The model under review builds one solid part; all positions refer to its coordinate system, in mm. A direction names the side the tool comes from. Round coordinates to 2 decimals unless told otherwise and drop trailing zeros. Order: outer loops, then holes, each group sorted by start corner. A loop starts at its lowest first (then second) coordinate and runs counter-clockwise, first axis right, second up.
1) Clearance check with flat-ended pins moving along their axes: P1, Ø4, axis at x = -2.5, y = -13, coming from the +Z side; P2, Ø5, axis at x = 3, y = -13, coming from the +Z side; P3, Ø3, axis at x = 6, z = 5.2, coming from the -Y side. State where each tip first meets the part, or that it passes through.
2) Consider section B-B (z = 5.2). Give the boundary of the cut face in (x, y), then the cut area to 3 significant figures.
3) Consider section C-C (y = 17.5). Give the boundary of the cut face in (x, z), then the cut area to 3 significant figures.
4) Consider section D-D (x = -14.5). Give the boundary of the cut face in (y, z), then the cut area to 3 significant figures.
5) Machinability: for faces 1 (the face through (5, -9, 0)), 2 (the face through (0, -15.2, 6)), 3 (the face through (4.78, 18.3, 5.47)), 4 (the face through (-0.2, 15.5, 7.7)), which of the approach directions +Z, -Z, +X, -X, +Y, -Y give a long, thin tool a straight path to every point of the face, cutting with its end or side? Answer none if there is none.
6) Mouldability with a two-part tool opening along X and no side actions: class faces 5 (the face through (0.2, -15.4, 7.7)), 6 (the face through (20.32, -8.43, 1.76)), 7 (the face through (0, 15.2, 6)) as pulls with the +X half, pulls with the -X half, needs draft (parallel to the pull), parting line crosses it, or undercut.
7) Consider section A-A (z = 9.25). Give the boundary of the cut face in (x, y).
8) To check wall thickness, follow L1, parallel to Y at x = 0, z = 3; L2, parallel to Y at x = 0, z = 2; L3, parallel to Z at x = 6, y = 19. State the ranges of each line that lie inside material, in increasing order.
from build123d import *

# Parameters (mm, degrees)
SKETCH1_R           = 22
BOSS_EXTRUDE1_DEPTH = 11
SKETCH2_R           = 20.05
CUT_EXTRUDE1_DEPTH  = 8.3
SKETCH3_W           = 67.682797152
SKETCH3_H           = 30.4
CUT_EXTRUDE2_DEPTH  = 8.3
SKETCH4_R           = 1.75
CUT_EXTRUDE3_DEPTH  = 5
CIRPATTERN1_COUNT   = 2
CUT_EXTRUDE4_REACH  = 35
SKETCH5_R           = 9
CHAMFER1_SIZE       = 1.5
CHAMFER2_SIZE       = 0.5
SKETCH6_OUTSIDE_W   = 58.638
SKETCH6_OUTSIDE_H   = 58.638
SKETCH6_OUTSIDE_W_2 = 90.952157774
SKETCH6_OUTSIDE_H_2 = 47
CUT_EXTRUDE5_DEPTH  = 8.3
BOSS_EXTRUDE2_START = 5
SKETCH7_R           = 1.75
BOSS_EXTRUDE2_DEPTH = 5
SKETCH8_R           = 1.25
CUT_EXTRUDE6_DEPTH  = 11


with BuildPart() as part:
    # Sketch1 → Boss-Extrude1 (new body)
    with BuildSketch(Plane.XY):
        Circle(SKETCH1_R)
    extrude(amount=BOSS_EXTRUDE1_DEPTH)

    # Sketch2 → Cut-Extrude1 (cut)
    with BuildSketch(Plane.XY.offset(11)):
        Circle(SKETCH2_R)
    extrude(amount=-CUT_EXTRUDE1_DEPTH, mode=Mode.SUBTRACT)

    # Sketch3 → Cut-Extrude2 (cut)
    with BuildSketch(Plane.XY.offset(2.7)):
        Rectangle(SKETCH3_W, SKETCH3_H)
    extrude(amount=CUT_EXTRUDE2_DEPTH, mode=Mode.SUBTRACT)

    # Sketch4 → Cut-Extrude3 (cut)
    with BuildSketch(Plane(origin=(0, 0, 0), x_dir=(-1, 0, 0), z_dir=(0, 0, -1))):
        with Locations((0, 17.5)):
            Circle(SKETCH4_R)
    cut_extrude3 = extrude(amount=-CUT_EXTRUDE3_DEPTH, mode=Mode.SUBTRACT)

    # CirPattern1: Cut-Extrude3 ×2 about axis
    cirpattern1_axis = Axis((0, 0, 0), (0, 0, 1))
    for i in range(1, CIRPATTERN1_COUNT):
        add(cut_extrude3.rotate(cirpattern1_axis, i * 360 / CIRPATTERN1_COUNT), mode=Mode.SUBTRACT)

    # Sketch5 → Cut-Extrude4 (cut, up to next)
    with BuildSketch(Plane(origin=(0, 0, 0), x_dir=(-1, 0, 0), z_dir=(0, 0, -1)), mode=Mode.PRIVATE) as cut_extrude4_sk1:
        Circle(SKETCH5_R)
    cut_extrude4_tool1 = extrude(cut_extrude4_sk1.sketch, amount=-CUT_EXTRUDE4_REACH, mode=Mode.PRIVATE) & part.part
    add(cut_extrude4_tool1.solids().sort_by_distance((0, 0, 0))[0], mode=Mode.SUBTRACT)

    # Chamfer1
    chamfer1_edges = [part.edges().sort_by_distance(p)[0] for p in [
        (1.75, 17.5, 0),
        (-1.75, -17.5, 0),
    ]]
    chamfer(chamfer1_edges, length=CHAMFER1_SIZE)

    # Chamfer2
    chamfer2_edges = [part.edges().sort_by_distance(p)[0] for p in [
        (9, 0, 0),
    ]]
    chamfer(chamfer2_edges, length=CHAMFER2_SIZE)

    # Sketch6 outside → Cut-Extrude5 (cut)
    with BuildSketch(Plane.XY.offset(11)):
        Rectangle(SKETCH6_OUTSIDE_W, SKETCH6_OUTSIDE_H)
        Rectangle(SKETCH6_OUTSIDE_W_2, SKETCH6_OUTSIDE_H_2, mode=Mode.SUBTRACT)
    extrude(amount=-CUT_EXTRUDE5_DEPTH, mode=Mode.SUBTRACT)

    # Sketch7 → Boss-Extrude2 (add)
    # profile 1 of 2: a face of its own
    with BuildSketch(Plane.XY.offset(2.7).offset(BOSS_EXTRUDE2_START)):
        with BuildLine():
            Line((-13.075262904, 15.2), (13.075262904, 15.2))
            ThreePointArc((13.075262904, 15.2), (0, 20.05), (-13.075262904, 15.2))
        make_face()
        with Locations((0, 17.5)):
            Circle(SKETCH7_R, mode=Mode.SUBTRACT)
    # profile 2 of 2: a face of its own
    with BuildSketch(Plane.XY.offset(2.7).offset(BOSS_EXTRUDE2_START)):
        with BuildLine():
            Line((-13.075262904, -15.2), (13.075262904, -15.2))
            ThreePointArc((13.075262904, -15.2), (0, -20.05), (-13.075262904, -15.2))
        make_face()
        with Locations((0, -17.5)):
            Circle(SKETCH7_R, mode=Mode.SUBTRACT)
    extrude(amount=-BOSS_EXTRUDE2_DEPTH)

    # Sketch8 → Cut-Extrude6 (cut)
    with BuildSketch(Plane.XZ.offset(-15.2)):
        with Locations(Location((6, 5.2, 0), (0, 0, 270))):
            Circle(SKETCH8_R)
    extrude(amount=-CUT_EXTRUDE6_DEPTH, mode=Mode.SUBTRACT)


solid = part.part
Answer below:
1. P1: stops at z = 2.7
1. P2: stops at z = 7.7
1. P3: stops at y = -21.53
2. outline: (-15.9, -15.2) arc R22 ccw to (15.9, -15.2) - close; (-15.9, 15.2) - (4.75, 15.2) - (4.75, 21.48) arc R22 ccw to start; (7.25, 15.2) - (15.9, 15.2) arc R22 ccw to (7.25, 20.77) - close; hole circle Ø3.5 at (0, -17.5); hole circle Ø3.5 at (0, 17.5)
2. area: 265 mm2
3. outline: (-13.33, 0) - (-3.25, 0) - (-1.75, 1.5) - (-1.75, 7.7) - (-9.79, 7.7) - (-9.79, 11) - (-13.33, 11) - close; (1.75, 1.5) - (3.25, 0) - (13.33, 0) - (13.33, 11) - (9.79, 11) - (9.79, 7.7) - (1.75, 7.7) - close; hole circle Ø2.5 at (6, 5.2)
3. area: 195 mm2
4. outline: (-16.55, 0) - (16.55, 0) - (16.55, 11) - (15.2, 11) - (15.2, 2.7) - (-15.2, 2.7) - (-15.2, 11) - (-16.55, 11) - close
4. area: 112 mm2
5. face 1: -Z, +X, -X, +Y, -Y
5. face 2: +Z, +X, -X
5. face 3: +Y
5. face 4: +Z
6. face 5: undercut
6. face 6: parting line crosses it
6. face 7: needs draft
7. outline: (-15.9, -15.2) arc R22 ccw to (15.9, -15.2) - (13.08, -15.2) arc R20.05 cw to (-13.08, -15.2) - close; (-15.9, 15.2) - (-13.08, 15.2) arc R20.05 cw to (13.08, 15.2) - (15.9, 15.2) arc R22 ccw to start
8. L1: y = -22 to -19.25, -15.75 to -15.2, 15.2 to 15.75, 19.25 to 22
8. L2: y = -22 to -19.25, -15.75 to -9, 9 to 15.75, 19.25 to 22
8. L3: z = 0 to 3.95, 6.45 to 7.7
